Work out the finished part from the listing and answer in its coordinate system (mm). A direction names the side the tool comes from. Coordinates: 2 decimals unless noted, no trailing zeros. Order: outer loops, then holes, each group sorted by start corner. A loop starts at its lowest first (then second) coordinate and runs counter-clockwise, first axis right, second up. Notation, with made-up numbers: M -37.75,86.5 L 9.25,86.5 A26 cw 9.25,107.5 Z; hole C 1.5,65.25 d2. An arc over 180 degrees is marked long. Write item = value, one per line. Start each with the question number.
Q1. Each of these flat-tipped pins is pushed along its axis until it touches: P1, Ø1, axis at x = -115, z = -84, coming from the +Y side; P2, Ø3, axis at y = -161, z = -125, coming from the +X side; P3, Ø8, axis at y = 126.5, z = -166.5, coming from the +X side. Where does it stop, or does it pass through?
Q2. A tool of negligible diameter and unlimited length cuts with its end or side. For faces 4 (the cylindrical face through (3.255, -275.213, -189.44)), 5 (the cylindrical face through (-49.86, -224.53, -73.95)), from which of +Z, -Z, +X, -X, +Y, -Y can it reach the whole face along a straight path? Write none if from no direction.
Q3. Determine the mould class of faces 1 (the cylindrical face through (257.96, 236.55, -189.44)), 2 (the cylindrical face through (3.255, 324.787, -189.44)), 3 (the flat face through (5, 5, -230)) for opening direction X: released by +X, released by -X, zero draft, split by the parting line, or undercut.
Q4. Find section C-C on y = 0. Give the vertices of the cut face in (x, z), and give its area (3 significant figures).
Q5. Find section B-B on x = 268.5. Give the vertices of the cut face in (y, z).
Q6. Straight lines are drawn through the part: line 1 along Y through (x, z) = (0, -174); line 2 along X through (y, z) = (-150, -197); line 3 along Y through (x, z) = (-273, -166). For each, find the intervals that lie inside material, in ascending order.
Q7. Find section D-D on y = 300. Give the vertices of the cut face in (x, z), and give its area (3 significant figures).
Q8. Find section A-A on z = -70. Give the vertices of the cut face in (x, y), and give its area (3 significant figures).
```python
from build123d import *

# Parameters (mm, degrees)
SKETCH1_R               = 230
BOSS_EXTRUDE1_DEPTH     = 150
SKETCH2_R               = 350
BOSS_EXTRUDE2_DEPTH     = 80
CUT_EXTRUDE1_DEPTH      = 256
CUT_EXTRUDE1_DEPTH_BACK = 269
SKETCH3_R               = 25


with BuildPart() as part:
    # Sketch1 → Boss-Extrude1 (new body)
    with BuildSketch(Plane.XY):
        Circle(SKETCH1_R)
        with BuildLine():
            Line((-50, 141.421356237), (-50, 176.421356237))
            Line((-50, 176.421356237), (50, 176.421356237))
            Line((50, 176.421356237), (50, 141.421356237))
            ThreePointArc((50, 141.421356237), (0, -150), (-50, 141.421356237))
        make_face(mode=Mode.SUBTRACT)
    extrude(amount=-BOSS_EXTRUDE1_DEPTH)

    # Sketch2 → Boss-Extrude2 (add)
    with BuildSketch(Plane(origin=(0, 0, -150), x_dir=(-1, 0, 0), z_dir=(0, 0, -1))):
        Circle(SKETCH2_R)
    extrude(amount=BOSS_EXTRUDE2_DEPTH)

    # Sketch3 → Cut-Extrude1 (cut, two sides: drawn at the far end of the back side and taken through both)
    with BuildSketch(Plane(origin=(0, 0, -230), x_dir=(-1, 0, 0), z_dir=(0, 0, -1)).offset(-CUT_EXTRUDE1_DEPTH_BACK)):
        with Locations((0, 300)):
            Circle(SKETCH3_R)
        with Locations((259.807621135, 150)):
            Circle(SKETCH3_R)
        with Locations((259.807621135, -150)):
            Circle(SKETCH3_R)
        with Locations((0, -300)):
            Circle(SKETCH3_R)
        with Locations((-259.807621135, -150)):
            Circle(SKETCH3_R)
        with Locations((-259.807621135, 150)):
            Circle(SKETCH3_R)
    extrude(amount=CUT_EXTRUDE1_DEPTH + CUT_EXTRUDE1_DEPTH_BACK, mode=Mode.SUBTRACT)


solid = part.part
```
Findings below:
q1.P1 = 199.47
q1.P2 = 165.71
q1.P3 = 327.86
q2.face_4 = +Z, -Z
q2.face_5 = +Z
q3.face_1 = split by the parting line
q3.face_2 = undercut
q3.face_3 = zero draft
q4.outline = M -350,-230 L 350,-230 L 350,-150 L 230,-150 L 230,0 L 150,0 L 150,-150 L -150,-150 L -150,0 L -230,0 L -230,-150 L -350,-150 Z
q4.area = 80,000 mm^2
q5.outline = M -224.52,-230 L -173.44,-230 L -173.44,-150 L -224.52,-150 Z; M -126.56,-230 L 126.56,-230 L 126.56,-150 L -126.56,-150 Z; M 173.44,-230 L 224.52,-230 L 224.52,-150 L 173.44,-150 Z
q6.line_1 = -350 to -325, -275 to 275, 325 to 350
q6.line_2 = -316.23 to -284.81, -234.81 to 234.81, 284.81 to 316.23
q6.line_3 = -219.02 to -171.24, -128.76 to 128.76, 171.24 to 219.02
q7.outline = M -180.28,-230 L -25,-230 L -25,-150 L -180.28,-150 Z; M 25,-230 L 180.28,-230 L 180.28,-150 L 25,-150 Z
q7.area = 24,800 mm^2
q8.outline = C 0,0 d460; hole M -50,141.42 A150 ccw long 50,141.42 L 50,176.42 L -50,176.42 Z
q8.area = 92,600 mm^2
